```python
from build123d import *

# Parameters (mm, degrees)
BASE_BODY_DEPTH       = 50
BACK_WALL_SKETCH_W    = 80
BACK_WALL_SKETCH_H    = 24
BACK_WALL_DEPTH       = 50
WALL_NOTCH_SKETCH_W   = 60
WALL_NOTCH_SKETCH_H   = 14
WALL_NOTCH_CUT_DEPTH  = 120.899958299
SLOT_BOSS_DEPTH       = 26
SLOT_CUT_14MM_DEPTH   = 107.77078252
RIB_SKETCH_W          = 10
RIB_SKETCH_H          = 27
REINFORCING_RIB_DEPTH = 26
TRIM_CUT_DEPTH        = 84.815273071
TRIM_CUT_DEPTH_BACK   = 26


with BuildPart() as part:
    # Base Profile Sketch → Base Body (new body)
    with BuildSketch(Plane.XY):
        Polygon((0, 0), (40, 0), (80, 0), (80, -24), (70, -24), (70, -10), (10, -10), (10, -24), (0, -24), align=None)
    extrude(amount=-BASE_BODY_DEPTH)

    # Back Wall Sketch → Back Wall (add)
    with BuildSketch(Plane(origin=(0, 0, 0), x_dir=(1, 0, 0), z_dir=(0, 1, 0))):
        with Locations((40, 38)):
            Rectangle(BACK_WALL_SKETCH_W, BACK_WALL_SKETCH_H)
    extrude(amount=BACK_WALL_DEPTH)

    # Wall Notch Sketch → Wall Notch Cut (cut, through all)
    with BuildSketch(Plane(origin=(0, 50, 0), x_dir=(1, 0, 0), z_dir=(0, 1, 0))):
        with Locations((40, 43)):
            Rectangle(WALL_NOTCH_SKETCH_W, WALL_NOTCH_SKETCH_H)
    extrude(amount=-WALL_NOTCH_CUT_DEPTH, mode=Mode.SUBTRACT)

    # Slot Boss Sketch → Slot Boss (add)
    with BuildSketch(Plane.XY):
        with BuildLine():
            Line((26, 10), (26, -10))
            ThreePointArc((26, -10), (40, -24), (54, -10))
            Line((54, -10), (54, 10))
            ThreePointArc((54, 10), (40, 24), (26, 10))
        make_face()
    extrude(amount=-SLOT_BOSS_DEPTH)

    # Slot Sketch → Slot Cut 14mm (cut, through all)
    with BuildSketch(Plane.XY):
        with BuildLine():
            Line((33, -10), (33, 10))
            ThreePointArc((33, 10), (40, 17), (47, 10))
            Line((47, 10), (47, -10))
            ThreePointArc((47, -10), (40, -17), (33, -10))
        make_face()
    extrude(amount=-SLOT_CUT_14MM_DEPTH, mode=Mode.SUBTRACT)

    # Rib Sketch → Reinforcing Rib (add)
    with BuildSketch(Plane.XY.offset(-26)):
        with Locations((40, 36.5)):
            Rectangle(RIB_SKETCH_W, RIB_SKETCH_H)
    extrude(amount=REINFORCING_RIB_DEPTH)

    # Trim Line Sketch → Trim Cut (cut, two sides: drawn at the far end of the back side and taken through both)
    with BuildSketch(Plane.ZY.offset(-35).offset(-TRIM_CUT_DEPTH_BACK)):
        Polygon((-141.918286791, 170.034737621), (-26, 50), (0, 23.076696831), (115.918286791, -96.95804079), (355.987762032, 134.878532791), (98.151188451, 401.871311202), align=None)
    extrude(amount=TRIM_CUT_DEPTH + TRIM_CUT_DEPTH_BACK, mode=Mode.SUBTRACT)


solid = part.part
```
The listing builds one solid part. Answer for the finished solid, in the listing's coordinates (mm). A direction names the side the tool comes from. Round coordinates to 2 decimals unless told otherwise and drop trailing zeros. Loops run counter-clockwise (first coordinate to the right, second up) from the corner with the lowest first, then second, coordinate; pieces in that order, holes last.
1) A cutting plane is placed at D-D on z = -30.5. Determine the outline of the cut face in (x, y), plus the area to 3 significant figures.
Outcome:
outline: (0, -24) - (10, -24) - (10, -10) - (33, -10) - (33, 10) arc R7 cw to (47, 10) - (47, -10) - (70, -10) - (70, -24) - (80, -24) - (80, 50) - (0, 50) - close
area: 4,720 mm2
2) For faces 5 (the face through (75, 12, -50)), 6 (the face through (13, 0, -13)), 7 (the face through (40, -18, -26)), 8 (the face through (51.6, 17.84, -12.82)), determine the directions among +Z, -Z, +X, -X, +Y, -Y from which every point of the face is accessible in a straight line to the end or side of a thin tool.
Outcome:
face 5: -Z, +X, -X, +Y, -Y
face 6: +Z, -X, +Y
face 7: -Z, -Y
face 8: +Z, +X, +Y
3) A cutting plane is placed at A-A on z = -40. Determine the outline of the cut face in (x, y).
Outcome:
outline: (0, -24) - (10, -24) - (10, 50) - (0, 50) - close; (70, -24) - (80, -24) - (80, 50) - (70, 50) - close
4) A cutting plane is placed at B-B on x = 40. Determine the outline of the cut face in (y, z), plus the area to 3 significant figures.
Outcome:
outline: (-24, -26) - (-17, -26) - (-17, 0) - (-24, 0) - close; (17, -36) - (50, -36) - (50, -26) - (23.08, 0) - (17, 0) - close
area: 1,020 mm2
5) A cutting plane is placed at C-C on y = 6.5. Determine the outline of the cut face in (x, z), plus the area to 3 significant figures.
Outcome:
outline: (0, -50) - (10, -50) - (10, -36) - (33, -36) - (33, 0) - (26, 0) - (26, -26) - (0, -26) - close; (47, -36) - (70, -36) - (70, -50) - (80, -50) - (80, -26) - (54, -26) - (54, 0) - (47, 0) - close
area: 1,300 mm2
6) Consider line 1 (X direction, y = 29.5, z = -43.5); line 2 (X direction, y = 8.5, z = -14); line 3 (X direction, y = -11.5, z = -20.5). Determine where each line is inside the solid, lowest interval first.
Outcome:
line 1: x = 0 to 10, 70 to 80
line 2: x = 26 to 33, 47 to 54
line 3: x = 0 to 10, 26.08 to 33.16, 46.84 to 53.92, 70 to 80
7) For a pull along Y with two mould halves and no side action, classify faces 1 (the face through (61, -10, -18)), 2 (the face through (40, 17, -18)), 3 (the face through (48, -5, 0)), 4 (the face through (40, -17, -13)) as released by +Y, released by -Y, zero draft, split by the parting line, or undercut.
Outcome:
face 1: released by -Y
face 2: undercut
face 3: zero draft
face 4: undercut
8) Given P1, Ø11, axis at x = 38, y = -19, coming from the -Z side; P2, Ø6, axis at y = 1, z = -15, coming from the -X side; P3, Ø10, axis at x = 40, y = 31, coming from the -Z side; P4, Ø11.5, axis at x = 57.5, z = -14, coming from the -Y side, each flat-ended and moving along its own axis, determine where each tip first touches the part or whether it passes through.
Outcome:
P1: stops at z = -26
P2: stops at x = 0
P3: stops at z = -36
P4: stops at y = -17.61
